Source: CAD feature listing. Evaluate the final solid. Frame: model axes, mm. Give positions to 0.01 mm unless a question says otherwise; leave off trailing zeros. Order: outer loops, then holes, each group sorted by start corner. A loop starts at its lowest first (then second) coordinate and runs counter-clockwise, first axis right, second up. Notation, with made-up numbers: M 86.25,44 L 126.25,44 A14 ccw 126.25,71 Z; hole C 81.25,53 d6. An arc over 180 degrees is marked long. Return JSON: item names as keys, results as strings.
from build123d import *

# Parameters (mm, degrees)
SKETCH1_R           = 50
BOSS_EXTRUDE1_DEPTH = 5
SKETCH2_R           = 1.9
CUT_EXTRUDE1_DEPTH  = 71.887234394
CIRPATTERN1_COUNT   = 4
SKETCH3_R           = 17.5
CUT_EXTRUDE2_DEPTH  = 71.887234394
CIRPATTERN2_COUNT   = 4
SKETCH4_R           = 8
SKETCH4_R_2         = 3
SKETCH4_R_3         = 2.5
SKETCH4_R_4         = 2
CUT_EXTRUDE3_DEPTH  = 71.887234394
CIRPATTERN3_COUNT   = 4


with BuildPart() as part:
    # Sketch1 → Boss-Extrude1 (new body)
    with BuildSketch(Plane.XY):
        Circle(SKETCH1_R)
    extrude(amount=BOSS_EXTRUDE1_DEPTH)

    # Sketch2 → Cut-Extrude1 (cut, through all)
    with BuildSketch(Plane(origin=(0, 0, 0), x_dir=(-1, 0, 0), z_dir=(0, 0, -1))):
        with Locations((-5.656854249, 5.656854249)):
            Circle(SKETCH2_R)
    cut_extrude1 = extrude(amount=-CUT_EXTRUDE1_DEPTH, mode=Mode.SUBTRACT)

    # CirPattern1: Cut-Extrude1 ×4 about axis
    cirpattern1_axis = Axis((0, 0, 0), (0, 0, 1))
    for i in range(1, CIRPATTERN1_COUNT):
        add(cut_extrude1.rotate(cirpattern1_axis, i * 360 / CIRPATTERN1_COUNT), mode=Mode.SUBTRACT)

    # Sketch3 → Cut-Extrude2 (cut, through all)
    with BuildSketch(Plane(origin=(0, 0, 0), x_dir=(-1, 0, 0), z_dir=(0, 0, -1))):
        with Locations((0, 30)):
            Circle(SKETCH3_R)
    cut_extrude2 = extrude(amount=-CUT_EXTRUDE2_DEPTH, mode=Mode.SUBTRACT)

    # CirPattern2: Cut-Extrude2 ×4 about axis
    cirpattern2_axis = Axis((0, 0, 0), (0, 0, 1))
    for i in range(1, CIRPATTERN2_COUNT):
        add(cut_extrude2.rotate(cirpattern2_axis, i * 360 / CIRPATTERN2_COUNT), mode=Mode.SUBTRACT)

    # Sketch4 → Cut-Extrude3 (cut, through all)
    with BuildSketch(Plane(origin=(0, 0, 0), x_dir=(-1, 0, 0), z_dir=(0, 0, -1))):
        with Locations((-28.284271247, 28.284271247)):
            Circle(SKETCH4_R)
        with Locations((-18.686291501, 18.686291501)):
            Circle(SKETCH4_R_2)
        with Locations((-13.736544033, 13.736544033)):
            Circle(SKETCH4_R_3)
        with Locations((-9.493903346, 9.493903346)):
            Circle(SKETCH4_R_4)
        with Locations((-20.231783609, 40.939603832)):
            Circle(SKETCH4_R_4)
        with Locations((-40.939603832, 20.231783609)):
            Circle(SKETCH4_R_4)
    cut_extrude3 = extrude(amount=-CUT_EXTRUDE3_DEPTH, mode=Mode.SUBTRACT)

    # CirPattern3: Cut-Extrude3 ×4 about axis
    cirpattern3_axis = Axis((0, 0, 0), (0, 0, 1))
    for i in range(1, CIRPATTERN3_COUNT):
        add(cut_extrude3.rotate(cirpattern3_axis, i * 360 / CIRPATTERN3_COUNT), mode=Mode.SUBTRACT)


solid = part.part
1. Draft query along X for faces 1 (the face through (47.69, 15.02, 2.46)), 2 (the face through (0, -3, 0)), 3 (the face through (-36.216, 29.326, 2.465)). Return one class per face: pulls with the +X half, pulls with the -X half, needs draft (parallel to the pull), parting line crosses it, or undercut.
Evaluation:
{"face 1": "parting line crosses it", "face 2": "needs draft", "face 3": "undercut"}
2. Ray query, probe 1 along Y at (x, z) = (0, 3); probe 2 along X at (y, z) = (9, 4.85); probe 3 along Y at (x, z) = (10.5, 0.45). Return the intervals inside material, ascending.
Evaluation:
{"probe 1": "y = -50 to -47.5, -12.5 to 12.5, 47.5 to 50", "probe 2": "x = -49.18 to -45.01, -14.99 to -11.43, -7.56 to 7.56, 11.43 to 14.99, 45.01 to 49.18", "probe 3": "y = -48.89 to -44, -16 to -11.22, -7.77 to 7.77, 11.22 to 16, 44 to 48.89"}
3. First-contact query: pin 1 (1.5 mm diameter, centred on x = 35, z = 0.5, fed in from +Y). Flat tip, straight axial feed; report the tip coordinate or a pass-through.
Evaluation:
{"pin 1": "stops at y = 36.43"}
4. Section query A-A (x = 0). Return loops of the section in (y, z).
Evaluation:
{"outline": "M -50,0 L -47.5,0 L -47.5,5 L -50,5 Z; M -12.5,0 L 12.5,0 L 12.5,5 L -12.5,5 Z; M 47.5,0 L 50,0 L 50,5 L 47.5,5 Z"}
5. Section query D-D (x = -32). Return loops of the section in (y, z), then the cut area to 3 significant figures.
Evaluation:
{"outline": "M -38.42,0 L -35.37,0 L -35.37,5 L -38.42,5 Z; M -21.2,0 L -17.39,0 L -17.39,5 L -21.2,5 Z; M 17.39,0 L 21.2,0 L 21.2,5 L 17.39,5 Z; M 35.37,0 L 38.42,0 L 38.42,5 L 35.37,5 Z", "area": "68.6 mm^2"}
6. Section query C-C (y = 27). Return loops of the section in (x, z).
Evaluation:
{"outline": "M -42.08,0 L -36.18,0 L -36.18,5 L -42.08,5 Z; M -20.39,0 L -17.24,0 L -17.24,5 L -20.39,5 Z; M 17.24,0 L 20.39,0 L 20.39,5 L 17.24,5 Z; M 36.18,0 L 42.08,0 L 42.08,5 L 36.18,5 Z"}
